```python
from build123d import *

# Parameters (mm, degrees)
MAIN_BODY_DEPTH              = 12
UPPER_PLATE_SKETCH_W         = 50
UPPER_PLATE_SKETCH_H         = 50
UPPER_PLATE_DEPTH            = 12
WEB_BLOCK_DEPTH              = 12
PIN_HUB_BOSS_A_SKETCH_R      = 15
PIN_HUB_BOSS_A_SKETCH_R_2    = 7
PIN_HUB_BOSS_A_30_DEPTH      = 6
PIN_START                    = -62
PIN_BORE_SKETCH_R            = 7
PIN_BORE_14_DEPTH            = 62
PIN_START_2                  = 6
PIN_HUB_BOSS_B_SKETCH_R      = 15
PIN_HUB_BOSS_B_SKETCH_R_2    = 7
PIN_HUB_BOSS_B_30_DEPTH      = 6
FORK_LUG_DEPTH               = 12
FORK_HUB_SKETCH_R            = 12.5
FORK_HUB_25_DEPTH            = 19
FORK_BORE_SKETCH_R           = 9
FORK_BORE_18_DEPTH           = 101.304536288
FORK_START                   = -12
FORK_FILLER_BLOCK_SKETCH_R   = 12.5
FORK_FILLER_BLOCK_SKETCH_R_2 = 9
FORK_FILLER_BLOCK_DEPTH      = 12
FORK_START_2                 = 7
FORK_SPACER_RING_SKETCH_R    = 12.5
FORK_SPACER_RING_SKETCH_R_2  = 9
FORK_SPACER_RING_25_DEPTH    = 7


with BuildPart() as part:
    # Main Body Side Profile Sketch → Main Body (new body)
    with BuildSketch(Plane(origin=(0, 0, 0), x_dir=(0, 0, -1), z_dir=(1, 0, 0))):
        with BuildLine():
            Line((0, 0), (0, 50))
            Line((0, 50), (12, 50))
            Line((12, 50), (12, 44))
            Line((12, 44), (37, 44))
            Line((37, 44), (37, 50))
            Line((37, 50), (50, 50))
            ThreePointArc((50, 50), (75, 25), (50, 0))
            Line((50, 0), (37, 0))
            Line((37, 0), (37, 6))
            Line((37, 6), (12, 6))
            Line((12, 6), (12, 0))
            Line((12, 0), (0, 0))
        make_face()
    extrude(amount=MAIN_BODY_DEPTH)

    # Upper Plate Sketch → Upper Plate (add)
    with BuildSketch(Plane.XY):
        with Locations((-13, 25)):
            Rectangle(UPPER_PLATE_SKETCH_W, UPPER_PLATE_SKETCH_H)
    extrude(amount=-UPPER_PLATE_DEPTH)

    # Web Block Sketch → Web Block (add)
    with BuildSketch(Plane.ZY.offset(38)):
        with BuildLine():
            Line((-12, 44), (-37, 44))
            Line((-37, 44), (-37, 50))
            Line((-37, 50), (-50, 50))
            ThreePointArc((-50, 50), (-75, 25), (-50, 0))
            Line((-50, 0), (-37, 0))
            Line((-37, 0), (-37, 6))
            Line((-37, 6), (-12, 6))
            Line((-12, 6), (-12, 44))
        make_face()
    extrude(amount=-WEB_BLOCK_DEPTH)

    # Pin Hub Boss A Sketch → Pin Hub Boss A Ø30 (add)
    with BuildSketch(Plane(origin=(12, 0, 0), x_dir=(0, 0, -1), z_dir=(1, 0, 0))):
        with Locations(Location((50, 25, 0), (0, 0, 180))):
            Circle(PIN_HUB_BOSS_A_SKETCH_R)
        with Locations((50, 25)):
            Circle(PIN_HUB_BOSS_A_SKETCH_R_2, mode=Mode.SUBTRACT)
    extrude(amount=PIN_HUB_BOSS_A_30_DEPTH)

    # Pin Bore Sketch → Pin Bore Ø14 (cut)
    with BuildSketch(Plane(origin=(12, 0, 0), x_dir=(0, 0, -1), z_dir=(1, 0, 0)).offset(PIN_START)):
        with Locations(Location((50, 25, 0), (0, 0, 180))):
            Circle(PIN_BORE_SKETCH_R)
    extrude(amount=PIN_BORE_14_DEPTH, mode=Mode.SUBTRACT)

    # Pin Hub Boss B Sketch → Pin Hub Boss B Ø30 (add)
    with BuildSketch(Plane.ZY.offset(38).offset(PIN_START_2)):
        with Locations((-50, 25)):
            Circle(PIN_HUB_BOSS_B_SKETCH_R)
        with Locations((-50, 25)):
            Circle(PIN_HUB_BOSS_B_SKETCH_R_2, mode=Mode.SUBTRACT)
    extrude(amount=-PIN_HUB_BOSS_B_30_DEPTH)

    # Fork Lug Sketch → Fork Lug (add)
    with BuildSketch(Plane(origin=(0, 50, 0), x_dir=(1, 0, 0), z_dir=(0, 1, 0))):
        with BuildLine():
            Line((-38, 0), (-24.392972847, -30.142972847))
            ThreePointArc((-24.392972847, -30.142972847), (-13, -37.5), (-1.607027153, -30.142972847))
            Line((-1.607027153, -30.142972847), (12, 0))
            Line((12, 0), (-38, 0))
        make_face()
    extrude(amount=-FORK_LUG_DEPTH)

    # Fork Hub Sketch → Fork Hub Ø25 (add)
    with BuildSketch(Plane(origin=(0, 50, 0), x_dir=(1, 0, 0), z_dir=(0, 1, 0))):
        with Locations(Location((-13, -25, 0), (0, 0, 270))):
            Circle(FORK_HUB_SKETCH_R)
    extrude(amount=-FORK_HUB_25_DEPTH)

    # Fork Bore Sketch → Fork Bore Ø18 (cut, through all)
    with BuildSketch(Plane(origin=(0, 50, 0), x_dir=(1, 0, 0), z_dir=(0, 1, 0))):
        with Locations(Location((-13, -25, 0), (0, 0, 270))):
            Circle(FORK_BORE_SKETCH_R)
    extrude(amount=-FORK_BORE_18_DEPTH, mode=Mode.SUBTRACT)

    # Fork Filler Block Sketch → Fork Filler Block (add)
    # profile 1 of 2: a face of its own
    with BuildSketch(Plane.XZ.offset(FORK_START)):
        with BuildLine():
            Line((-24.392972847, 30.142972847), (-38, 0))
            Line((-38, 0), (12, 0))
            Line((12, 0), (-1.607027153, 30.142972847))
            ThreePointArc((-1.607027153, 30.142972847), (-0.779890332, 27.630383946), (-0.5, 25))
            ThreePointArc((-0.5, 25), (-15.630383946, 12.779890332), (-24.392972847, 30.142972847))
        make_face()
    # profile 2 of 2: a face of its own
    with BuildSketch(Plane.XZ.offset(FORK_START)):
        with Locations(Location((-13, 25, 0), (0, 0, 90))):
            Circle(FORK_FILLER_BLOCK_SKETCH_R)
        with Locations(Location((-13, 25, 0), (0, 0, 90))):
            Circle(FORK_FILLER_BLOCK_SKETCH_R_2, mode=Mode.SUBTRACT)
    extrude(amount=FORK_FILLER_BLOCK_DEPTH)

    # Fork Spacer Ring Sketch → Fork Spacer Ring Ø25 (add)
    with BuildSketch(Plane(origin=(0, 12, 0), x_dir=(1, 0, 0), z_dir=(0, 1, 0)).offset(FORK_START_2)):
        with Locations(Location((-13, -25, 0), (0, 0, 270))):
            Circle(FORK_SPACER_RING_SKETCH_R)
        with Locations(Location((-13, -25, 0), (0, 0, 270))):
            Circle(FORK_SPACER_RING_SKETCH_R_2, mode=Mode.SUBTRACT)
    extrude(amount=-FORK_SPACER_RING_25_DEPTH)


solid = part.part
```
Here's how the part is built. I have some questions about the finished solid (model axes, mm). A direction names the side the tool comes from. Give positions to 0.01 mm unless a question says otherwise; leave off trailing zeros. Order: outer loops, then holes, each group sorted by start corner. A loop starts at its lowest first (then second) coordinate and runs counter-clockwise, first axis right, second up. Notation, with made-up numbers: (-6, 30) -> (9, 30) arc R31 cw to (9, 56) -> close; hole circle Ø10 at (-31, 57). An arc over 180 degrees is marked (long way). Use CSV: the item, a comma, the result in double quotes. Start each with the question number.
Item 1: On a 3-axis mill with a long thin cutter (end or side, diameter ignored), from which of +Z, -Z, +X, -X, +Y, -Y can I reach the whole of each face in a straight line? I mean faces 1 (the flat face through (0, 20, -44)), 2 (the flat face through (6, 3, -37)), 3 (the flat face through (-13, 25, 0)), 4 (the flat face through (12, 25, -30)). Say none if no direction works.
Item 2: If I drill on probe 1 along Z at (x, y) = (-13, 16); probe 2 along X at (y, z) = (13, -68); probe 3 along X at (y, z) = (23, -59), over which ranges is the centre line in solid material (lowest first)? Write a range as [from, to].
Item 3: Suppose I cut it at B-B (y = 25). List the corners of the cut face in (x, z) for me.
Item 4: Suppose I cut it at A-A (z = -17). List the corners of the cut face in (x, y) for me, and give its area (3 significant figures).
Item 5: Suppose I cut it at C-C (x = -13). List the corners of the cut face in (y, z) for me.
Item 6: Thinking about a two-plate mould opening in X: for faces 5 (the flat face through (-26, 20, -44)), 6 (the flat face through (-38, 25, -29)), 7 (the flat face through (5.101, 44.084, 15.282)), 8 (the flat face through (-32, 44, -24)), which applies, pulls with the +X half, pulls with the -X half, needs draft (parallel to the pull), parting line crosses it, or undercut?
Item 7: I'm going to push flat-ended pins straight in: P1, Ø12, axis at x = -21.5, y = 5.5, coming from the +Z side; P2, Ø1, axis at x = -3.5, y = 11.5, coming from the +Z side; P3, Ø11, axis at y = 25, z = -50, coming from the +X side; P4, Ø9.5, axis at x = 7.5, z = -22.5, coming from the +Y side. Where does each tip first touch, or does it pass through?
Item 8: Suppose I cut it at D-D (y = 34). List the corners of the cut face in (x, z) for me.
Answer block:
1,face 1,"-Z, +Y, -Y"
1,face 2,"+X, -X, -Y"
1,face 3,"+X, -X"
1,face 4,"+X"
2,probe 1,"z = [-12, 0], [12.5, 16], [34, 37.5]"
2,probe 2,"x = [-38, -26], [0, 12]"
2,probe 3,"x = [-44, -26], [0, 18]"
3,outline,"(-44, -65) -> (-38, -65) -> (-38, -75) -> (-26, -75) -> (-26, -57) -> (-44, -57) -> close; (-44, -43) -> (-26, -43) -> (-26, -12) -> (0, -12) -> (0, -43) -> (18, -43) -> (18, -35) -> (12, -35) -> (12, 0) -> (-38, 0) -> (-38, -35) -> (-44, -35) -> close; (0, -75) -> (12, -75) -> (12, -65) -> (18, -65) -> (18, -57) -> (0, -57) -> close"
4,outline,"(-38, 6) -> (-26, 6) -> (-26, 44) -> (-38, 44) -> close; (0, 6) -> (12, 6) -> (12, 44) -> (0, 44) -> close"
4,area,"912 mm^2"
5,outline,"(0, -12) -> (50, -12) -> (50, 16) -> (31, 16) -> (31, 12.5) -> (38, 12.5) -> (38, 0) -> (12, 0) -> (12, 12.5) -> (19, 12.5) -> (19, 16) -> (0, 16) -> close; (0, 34) -> (19, 34) -> (19, 37.5) -> (0, 37.5) -> close; (31, 34) -> (50, 34) -> (50, 37.5) -> (31, 37.5) -> close"
6,face 5,"undercut"
6,face 6,"pulls with the -X half"
6,face 7,"pulls with the +X half"
6,face 8,"needs draft"
7,P1,"stops at z = 37.25"
7,P2,"stops at z = 33.67"
7,P3,"passes through"
7,P4,"stops at y = 44"
8,outline,"(-44, -62) -> (-38, -62) -> (-38, -73.32) -> (-26, -73.32) -> (-26, -12) -> (0, -12) -> (0, -73.32) -> (12, -73.32) -> (12, -62) -> (18, -62) -> (18, -38) -> (12, -38) -> (12, 0) -> (-38, 0) -> (-38, -38) -> (-44, -38) -> close; circle Ø25 at (-13, 25); hole circle Ø18 at (-13, 25)"
